from build123d import *

# Parameters (mm, degrees)
SKETCH_1_R      = 20
EXTRUDE_1_DEPTH = 64.4
SKETCH_2_W      = 3.325902221
SKETCH_2_H      = 1.7


with BuildPart() as part:
    # 草图1 → 凸台-拉伸1 (new body)
    with BuildSketch(Plane(origin=(0, 0, 0), x_dir=(1, 0, 0), z_dir=(0, 1, 0))):
        with Locations(Location((0, 0, 0), (0, 0, 270))):
            Circle(SKETCH_1_R)
    extrude(amount=EXTRUDE_1_DEPTH)

    # 草图2 → 切除-旋转1 (revolve, cut)
    with BuildSketch(Plane.XY, mode=Mode.PRIVATE) as cut_revolve_1_sk:
        with Locations((-20.41295111, 60.55)):
            Rectangle(SKETCH_2_W, SKETCH_2_H)
    cut_revolve_1 = revolve(cut_revolve_1_sk.sketch.rotate(Axis((0, 64.4, 0), (0, -1, 0)), 270), axis=Axis((0, 64.4, 0), (0, -1, 0)), mode=Mode.SUBTRACT)

    # 镜向1: 切除-旋转1 across plane
    add(cut_revolve_1.mirror(Plane(origin=(0, 32.2, 0), x_dir=(0, 0, 1), z_dir=(0, -1, 0))), mode=Mode.SUBTRACT)


solid = part.part
Work out the finished part from the listing and answer in its coordinate system (mm). A direction names the side the tool comes from. Round coordinates to 2 decimals unless told otherwise and drop trailing zeros. Write each loop counter-clockwise with the first axis right and the second up, starting at its lowest first coordinate (ties: lowest second). Pieces come first, ordered by that corner, then holes. Notation, with made-up numbers: M 56,11.25 L 67,11.25 A28 cw 67,35.25 Z; hole C -17,59.5 d4. An arc over 180 degrees is marked long. Use a Markdown table: item, result.
1) Determine the mould class of faces 3 (the face through (0, 64.4, 0)), 4 (the face through (18.304, 60.562, -4.065)), 5 (the face through (-19.524, 62.879, -4.336)) for opening direction Y: pulls with the +Y half, pulls with the -Y half, needs draft (parallel to the pull), parting line crosses it, or undercut.
Taken from the geometry:
| item | result |
|---|---|
| face 3 | pulls with the +Y half |
| face 4 | undercut |
| face 5 | needs draft |
2) The part is cut by section C-C on y = 17.5. Give the vertices of the cut face in (x, z), plus the area to 3 significant figures.
Taken from the geometry:
| item | result |
|---|---|
| outline | C 0,0 d40 |
| area | 1,260 mm2 |
3) Which of the six approach directions +Z, -Z, +X, -X, +Y, -Y give full straight-line access (tool end or side, diameter ignored) to faces 1 (the face through (-18, 4.7, 6)), 2 (the face through (0, 0, 0))?
Taken from the geometry:
| item | result |
|---|---|
| face 1 | none |
| face 2 | +Z, -Z, +X, -X, -Y |
4) Flat-ended cylindrical pins translate along their axes: pin 1 (20 mm diameter, centred on x = -4, z = 9.5, fed in from -Y); pin 2 (1 mm diameter, centred on y = 37.5, z = -4.5, fed in from +X); pin 3 (1 mm diameter, centred on y = 22, z = -12.5, fed in from +X); pin 4 (2 mm diameter, centred on y = 35, z = 1.5, fed in from +X). Find the tip coordinate at first contact, or state that the pin passes through.
Taken from the geometry:
| item | result |
|---|---|
| pin 1 | stops at y = 0 |
| pin 2 | stops at x = 19.6 |
| pin 3 | stops at x = 16 |
| pin 4 | stops at x = 19.99 |
5) Consider line 1 (Y direction, x = 17, z = -9); line 2 (Z direction, x = 7, y = 49.5) (3 decimals); line 3 (X direction, y = 35, z = 0). Determine where each line is inside the solid, lowest interval first. Write a range as [from, to].
Taken from the geometry:
| item | result |
|---|---|
| line 1 | y = [0, 3], [4.7, 59.7], [61.4, 64.4] |
| line 2 | z = [-18.735, 18.735] |
| line 3 | x = [-20, 20] |
6) The part is cut by section B-B on z = -3.5. Give the vertices of the cut face in (x, y).
Taken from the geometry:
| item | result |
|---|---|
| outline | M -19.69,0 L 19.69,0 L 19.69,3 L 18.42,3 L 18.42,4.7 L 19.69,4.7 L 19.69,59.7 L 18.42,59.7 L 18.42,61.4 L 19.69,61.4 L 19.69,64.4 L -19.69,64.4 L -19.69,61.4 L -18.42,61.4 L -18.42,59.7 L -19.69,59.7 L -19.69,4.7 L -18.42,4.7 L -18.42,3 L -19.69,3 Z |
7) The part is cut by section A-A on x = -8. Give the vertices of the cut face in (y, z).
Taken from the geometry:
| item | result |
|---|---|
| outline | M 0,-18.33 L 3,-18.33 L 3,-16.96 L 4.7,-16.96 L 4.7,-18.33 L 59.7,-18.33 L 59.7,-16.96 L 61.4,-16.96 L 61.4,-18.33 L 64.4,-18.33 L 64.4,18.33 L 61.4,18.33 L 61.4,16.96 L 59.7,16.96 L 59.7,18.33 L 4.7,18.33 L 4.7,16.96 L 3,16.96 L 3,18.33 L 0,18.33 Z |
